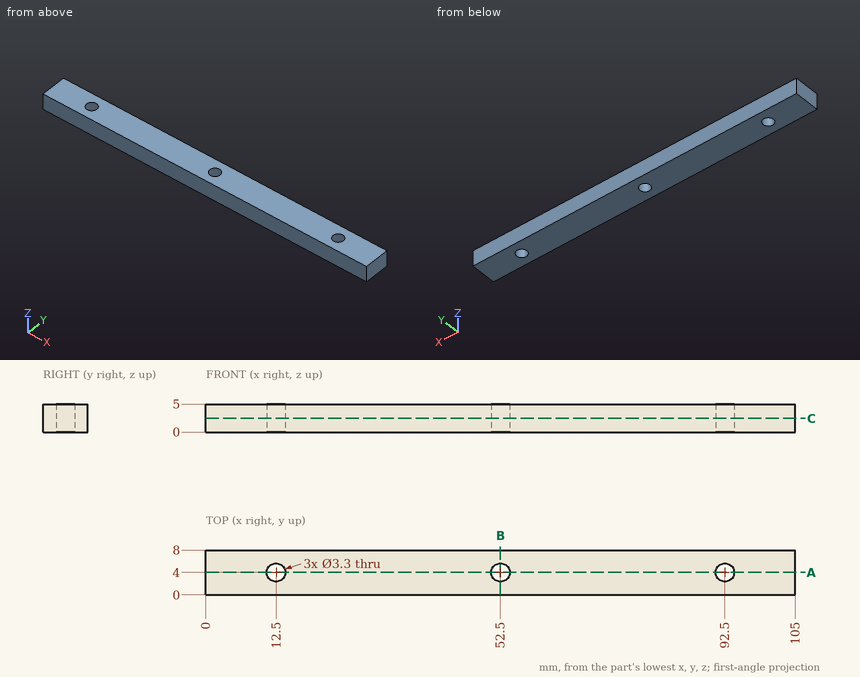
Verification items for this drawing (mm, ordinates from the low corner). Coordinates: 2 decimals unless noted, no trailing zeros. Order: outer loops, then holes, each group sorted by start corner. A loop starts at its lowest first (then second) coordinate and runs counter-clockwise, first axis right, second up. Notation, with made-up numbers: (57.5, -0.5) - (79.5, -0.5) arc R19 cw to (79.5, 13.5) - close; hole circle Ø10 at (2.25, 50). An arc over 180 degrees is marked (long way). Answer in a Markdown table with one row per item. Add a question column.
1. Section check B-B (x = 52.5). Enter the section's corners in (y, z).
2. Section check A-A (y = 4). Enter the section's corners in (x, z).
3. Section check C-C (z = 2.45). Enter the section's corners in (x, y).
4. Gauge pin test, flat ends, axial feed: pin 1 Ø1 at (x, y) = (82.5, 4.5) entering from -Z; pin 2 Ø2.5 at (x, y) = (52.5, 4) entering from -Z. Record the tip position at first contact, or that the pin passes through.
5. Material ranges on L1, parallel to Y at x = 92.5, z = 2.65; L2, parallel to X at y = 5.25, z = 2.5; L3, parallel to X at y = 3.5, z = 3, recorded low to high. Write a range as [from, to].
Data:
| question | item | result |
|---|---|---|
| 1 | outline | (0, 0) - (2.35, 0) - (2.35, 5) - (0, 5) - close; (5.65, 0) - (8, 0) - (8, 5) - (5.65, 5) - close |
| 2 | outline | (0, 0) - (10.85, 0) - (10.85, 5) - (0, 5) - close; (14.15, 0) - (50.85, 0) - (50.85, 5) - (14.15, 5) - close; (54.15, 0) - (90.85, 0) - (90.85, 5) - (54.15, 5) - close; (94.15, 0) - (105, 0) - (105, 5) - (94.15, 5) - close |
| 3 | outline | (0, 0) - (105, 0) - (105, 8) - (0, 8) - close; hole circle Ø3.3 at (12.5, 4); hole circle Ø3.3 at (52.5, 4); hole circle Ø3.3 at (92.5, 4) |
| 4 | pin 1 | stops at z = 0 |
| 4 | pin 2 | passes through |
| 5 | L1 | y = [0, 2.35], [5.65, 8] |
| 5 | L2 | x = [0, 11.42], [13.58, 51.42], [53.58, 91.42], [93.58, 105] |
| 5 | L3 | x = [0, 10.93], [14.07, 50.93], [54.07, 90.93], [94.07, 105] |
